Part model, mm, in its own coordinate system. Face numbers are marked on the shaded views. A direction names the side the tool comes from. Round coordinates to 2 decimals unless told otherwise and drop trailing zeros. Write each loop counter-clockwise with the first axis right and the second up, starting at its lowest first coordinate (ties: lowest second). Pieces come first, ordered by that corner, then holes. Notation, with made-up numbers: M 11.5,68 L 26.5,68 A21 cw 26.5,90 Z; hole C 18.5,-17.75 d5. An arc over 180 degrees is marked long. Use a Markdown table: item, result. Add a question column.
1) Slice it at B-B on y = 20. Write the cut outline in (x, z), plus the area to 3 significant figures.
2) Slice it at C-C on x = -4.5. Write the cut outline in (y, z), plus the area to 3 significant figures.
3) Slice it at D-D on y = 62. Write the cut outline in (x, z).
4) Slice it at A-A on z = 10.5. Write the cut outline in (x, y), plus the area to 3 significant figures.
5) Which spindle directions (+Z, -Z, +X, -X, +Y, -Y) get a long thin tool onto all of the face, cutting with end or side? Do the marked faces 5, 6, 7, 8 and 9. Say none if no direction does.
6) Drop flat-ended pins along their axis: P1, Ø16, axis at x = 30, y = 50, coming from the +Z side; P2, Ø13, axis at x = 21, y = 46, coming from the -Z side; P3, Ø6.5, axis at y = 25.5, z = -7, coming from the -X side; P4, Ø12, axis at x = -10.5, z = -18, coming from the -Y side. Give the stop position or say it passes through.
7) Wall check: probe 1 along Z at (x, y) = (25.5, 40.5); probe 2 along X at (y, z) = (3, 7); probe 3 along Z at (x, y) = (-23, 22.5). Give the ranges that are in metal, low to high.
8) Two-plate mould, pull along X, no slides. Class the marked faces 1, 2, 3 and 4: released by +X, released by -X, zero draft, split by the parting line, or undercut.
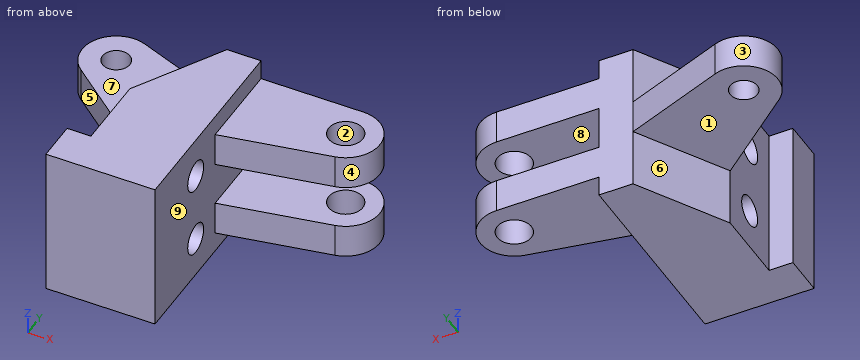
```python
from build123d import *

# Parameters (mm, degrees)
BASE_BLOCK_DEPTH           = 22.5
LUG_ARM_SKETCH_R           = 4
LUG_ARM_DEPTH              = 5
SIDE_HOLE_9_REACH          = 82.629
SIDE_HOLE_SKETCH_R         = 4.5
CLEVIS_FORK_SKETCH_R       = 5
CLEVIS_FORK_DEPTH          = 45
CLEVIS_PIN_HOLE_SKETCH_W   = 40
CLEVIS_PIN_HOLE_SKETCH_H   = 6
CLEVIS_PIN_HOLE_SKETCH_H_2 = 13
CLEVIS_PIN_HOLES_6_DEPTH   = 84.468772351


with BuildPart() as part:
    # Base Block Profile Sketch → Base Block (new, symmetric)
    with BuildSketch(Plane.XY):
        Polygon((0, 0), (-32, 0), (-32, 12), (-25.011106999, 12), (-25.011106999, 34), (-10, 60), (0, 60), align=None)
    extrude(amount=BASE_BLOCK_DEPTH, both=True)

    # Lug Arm Sketch → Lug Arm (add, symmetric)
    with BuildSketch(Plane.XY):
        with BuildLine():
            Line((-25.011106999, 34), (-49.811828564, 54.254815308))
            ThreePointArc((-49.811828564, 54.254815308), (-52.146569651, 67), (-39.941545389, 71.350647253))
            Line((-39.941545389, 71.350647253), (-10, 60))
            Line((-10, 60), (-25.011106999, 34))
        make_face()
        with Locations((-43.486315613, 62)):
            Circle(LUG_ARM_SKETCH_R, mode=Mode.SUBTRACT)
    extrude(amount=LUG_ARM_DEPTH, both=True)

    # Side Hole Sketch → Side Hole Ø9 (cut, up to next)
    with BuildSketch(Plane.ZY.offset(25.011106999), mode=Mode.PRIVATE) as side_hole_9_sk1:
        with Locations((10.5, 23)):
            Circle(SIDE_HOLE_SKETCH_R)
    side_hole_9_tool1 = extrude(side_hole_9_sk1.sketch, amount=-SIDE_HOLE_9_REACH, mode=Mode.PRIVATE) & part.part
    # Side Hole Sketch → Side Hole Ø9 (cut, up to next)
    with BuildSketch(Plane.ZY.offset(25.011106999), mode=Mode.PRIVATE) as side_hole_9_sk2:
        with Locations((-10.5, 23)):
            Circle(SIDE_HOLE_SKETCH_R)
    side_hole_9_tool2 = extrude(side_hole_9_sk2.sketch, amount=-SIDE_HOLE_9_REACH, mode=Mode.PRIVATE) & part.part
    add(side_hole_9_tool1.solids().sort_by_distance((-25.011107, 23, 10.5))[0], mode=Mode.SUBTRACT)
    add(side_hole_9_tool2.solids().sort_by_distance((-25.011107, 23, -10.5))[0], mode=Mode.SUBTRACT)

    # Clevis Fork Sketch → Clevis Fork (add)
    with BuildSketch(Plane.XY.offset(22.5)):
        with BuildLine():
            Line((0, 60), (30, 60))
            ThreePointArc((30, 60), (39.954230484, 50.95566494), (31.902581816, 40.182659096))
            Line((31.902581816, 40.182659096), (0, 34))
            Line((0, 34), (0, 60))
        make_face()
        with Locations((30, 50)):
            Circle(CLEVIS_FORK_SKETCH_R, mode=Mode.SUBTRACT)
    extrude(amount=-CLEVIS_FORK_DEPTH)

    # Clevis Pin Hole Sketch → Clevis Pin Holes Ø6 (cut, through all)
    with BuildSketch(Plane(origin=(0, 60, 0), x_dir=(1, 0, 0), z_dir=(0, 1, 0))):
        with Locations((20, -19.5)):
            Rectangle(CLEVIS_PIN_HOLE_SKETCH_W, CLEVIS_PIN_HOLE_SKETCH_H)
        with Locations((20, 0)):
            Rectangle(CLEVIS_PIN_HOLE_SKETCH_W, CLEVIS_PIN_HOLE_SKETCH_H_2)
        with Locations((20, 19.5)):
            Rectangle(CLEVIS_PIN_HOLE_SKETCH_W, CLEVIS_PIN_HOLE_SKETCH_H)
    extrude(amount=-CLEVIS_PIN_HOLES_6_DEPTH, mode=Mode.SUBTRACT)


solid = part.part
```
Entries:
| question | item | result |
|---|---|---|
| 1 | outline | M -25.01,-22.5 L 0,-22.5 L 0,-13.85 L -25.01,-13.85 Z; M -25.01,-7.15 L 0,-7.15 L 0,7.15 L -25.01,7.15 Z; M -25.01,13.85 L 0,13.85 L 0,22.5 L -25.01,22.5 Z |
| 1 | area | 790 mm^2 |
| 2 | outline | M 0,-22.5 L 60,-22.5 L 60,22.5 L 0,22.5 Z; hole C 23,-10.5 d9; hole C 23,10.5 d9 |
| 2 | area | 2,570 mm^2 |
| 3 | outline | M -53.49,-5 L -47.49,-5 L -47.49,5 L -53.49,5 Z; M -39.49,-5 L -15.28,-5 L -15.28,5 L -39.49,5 Z |
| 4 | outline | M -32,0 L 0,0 L 0,18.5 L -25.01,18.5 L -25.01,12 L -32,12 Z; M -25.01,27.5 L 0,27.5 L 0,34 L 31.9,40.18 A10 ccw 30,60 L -10,60 L -25.01,34 Z; hole C 30,50 d10 |
| 4 | area | 1,940 mm^2 |
| 5 | face 5 | +Z, -Z, -X |
| 5 | face 6 | -Z, -X, +Y |
| 5 | face 7 | +Z, -X, +Y |
| 5 | face 8 | +X, +Y, -Y |
| 5 | face 9 | +X, -Y |
| 6 | P1 | stops at z = 16.5 |
| 6 | P2 | stops at z = -16.5 |
| 6 | P3 | stops at x = -25.01 |
| 6 | P4 | stops at y = 0 |
| 7 | probe 1 | z = -16.5 to -6.5, 6.5 to 16.5 |
| 7 | probe 2 | x = -32 to 0 |
| 7 | probe 3 | z = -22.5 to -14.97, -6.03 to 6.03, 14.97 to 22.5 |
| 8 | face 1 | zero draft |
| 8 | face 2 | undercut |
| 8 | face 3 | split by the parting line |
| 8 | face 4 | released by +X |
